from build123d import *

# Parameters (mm, degrees)
SKETCH1_W                         = 120
SKETCH1_H                         = 12
SKETCH2_R                         = 85
BOSS_EXTRUDE1_DEPTH               = 2.5
SKETCH3_R                         = 80
BOSS_EXTRUDE2_DEPTH               = 3
F_12_5_12_5_DIAMETER_HOLE1_D      = 12.5
F_12_5_12_5_DIAMETER_HOLE1_DEPTH  = 14.5
M90_COUNTERBORE_HOLE1_D           = 100
M90_COUNTERBORE_HOLE1_CBORE_D     = 130
M90_COUNTERBORE_HOLE1_CBORE_DEPTH = 1
SKETCH8_R                         = 50.101943112
BOSS_EXTRUDE3_DEPTH               = 7


with BuildPart() as part:
    # Sketch1 → Revolve1 (revolve)
    with BuildSketch(Plane(origin=(0, 234.743963655, 0), x_dir=(1, 0, 0), z_dir=(0, 1, 0))):
        with Locations((581.230642584, 144.692981355)):
            Rectangle(SKETCH1_W, SKETCH1_H)
    revolve(axis=Axis((521.230642584, 234.743963655, -150.692981355), (0, 0, 1)))

    # Sketch2 → Boss-Extrude1 (add)
    with BuildSketch(Plane(origin=(0, 0, -150.692981355), x_dir=(-1, 0, 0), z_dir=(0, 0, -1))):
        with Locations((-521.230642584, 234.743963655)):
            Circle(SKETCH2_R)
    extrude(amount=BOSS_EXTRUDE1_DEPTH)

    # Sketch3 → Boss-Extrude2 (add)
    with BuildSketch(Plane.XY.offset(-138.692981355)):
        with Locations((521.230642584, 234.743963655)):
            Circle(SKETCH3_R)
    extrude(amount=BOSS_EXTRUDE2_DEPTH)

    # Ø12.5 (12.5) Diameter Hole1
    with Locations(Plane.XY.offset(-138.692981355)):
        with Locations((521.230642584, 337.243963655), (609.998246472, 285.993963655), (432.463038696, 285.993963655), (432.463038696, 183.493963655), (521.230642584, 132.243963655), (609.998246472, 183.493963655)):
            Hole(F_12_5_12_5_DIAMETER_HOLE1_D / 2, depth=F_12_5_12_5_DIAMETER_HOLE1_DEPTH)

    # M90 counterbore hole1 (through all)
    with Locations(Plane(origin=(0, 0, -153.192981355), x_dir=(-1, 0, 0), z_dir=(0, 0, -1))):
        with Locations((-521.230642584, 234.743963655)):
            CounterBoreHole(M90_COUNTERBORE_HOLE1_D / 2, M90_COUNTERBORE_HOLE1_CBORE_D / 2, M90_COUNTERBORE_HOLE1_CBORE_DEPTH)

    # Sketch8 → Boss-Extrude3 (add)
    with BuildSketch(Plane.XY.offset(-135.692981355)):
        with Locations((521.230642584, 234.743963655)):
            Circle(SKETCH8_R)
    extrude(amount=-BOSS_EXTRUDE3_DEPTH)


solid = part.part
Design review of the part built by this model. Coordinates are the model's own, in mm. A direction names the side the tool comes from. Coordinates: 2 decimals unless noted, no trailing zeros. Order: outer loops, then holes, each group sorted by start corner. A loop starts at its lowest first (then second) coordinate and runs counter-clockwise, first axis right, second up.
Item 1: For pin 1 Ø5 at (x, z) = (615.5, -146) entering from +Y; pin 2 Ø20 at (x, y) = (521.23, 337.24) entering from +Z; pin 3 Ø1 at (x, z) = (532.5, -140) entering from +Y, all flat-tipped, find the tip position at first contact; note any pin that passes through.
Item 2: For line 1 (X direction, y = 236.5, z = -152); line 2 (Z direction, x = 508, y = 244); line 3 (Z direction, x = 540, y = 291), list the stretches that pass through material, from the lowest coordinate up.
Item 3: The part is to be moulded in two halves that separate along Y. For faces 4 (the cylindrical face through (491.237, 177.078, -152.7)), 5 (the cylindrical face through (401.347, 240.02, -144.777)), 6 (the flat face through (520, 236, -135.693)), 7 (the cylindrical face through (429.1, 291.26, -144.78)), say which applies: pulls with the +Y half, pulls with the -Y half, needs draft (parallel to the pull), parting line crosses it, or undercut.
Item 4: Take a section at B-B, the plane z = -147.5. Write out the cut boundary in (x, y), then the cut area to 3 significant figures.
Item 5: Take a section at D-D, the plane y = 162. Write out the cut boundary in (x, z), then the cut area to 3 significant figures.
Item 6: For faces 1 (the flat face through (521, 235, -142.693)), 2 (the cylindrical face through (441.308, 238.261, -137.214)), 3 (the cylindrical face through (515.27, 339.12, -144.78)), list the 3-axis set-ups (+Z, -Z, +X, -X, +Y, -Y) from which the entire face can be reached by the end or side of a thin tool; tool diameter is ignored.
Item 7: Take a section at C-C, the plane x = 459. Write out the cut boundary in (y, z), then the cut area to 3 significant figures.
Item 8: Take a section at A-A, the plane x = 522. Write out the cut boundary in (y, z), then the cut area to 3 significant figures.
The answers:
1. pin 1: stops at y = 312.06
1. pin 2: stops at z = -138.69
1. pin 3: stops at y = 354.26
2. line 1: x = 436.25 to 471.26, 571.2 to 606.21
2. line 2: z = -142.69 to -135.69
2. line 3: z = -152.19 to -135.69
3. face 4: undercut
3. face 5: parting line crosses it
3. face 6: needs draft
3. face 7: undercut
4. outline: circle Ø240 at (521.23, 234.74); hole circle Ø12.5 at (432.46, 183.49); hole circle Ø12.5 at (432.46, 285.99); hole circle Ø100 at (521.23, 234.74); hole circle Ø12.5 at (521.23, 132.24); hole circle Ø12.5 at (521.23, 337.24); hole circle Ø12.5 at (610, 183.49); hole circle Ø12.5 at (610, 285.99)
4. area: 36,600 mm2
5. outline: (425.79, -150.69) - (477.26, -150.69) - (477.26, -153.19) - (565.2, -153.19) - (565.2, -150.69) - (616.67, -150.69) - (616.67, -138.69) - (554.52, -138.69) - (554.52, -135.69) - (487.94, -135.69) - (487.94, -138.69) - (425.79, -138.69) - close
5. area: 2,710 mm2
6. face 1: -Z
6. face 2: +Z
6. face 3: +Z, -Z
7. outline: (132.14, -150.69) - (176.84, -150.69) - (176.84, -153.19) - (215.97, -153.19) - (215.97, -152.19) - (253.51, -152.19) - (253.51, -153.19) - (292.64, -153.19) - (292.64, -150.69) - (337.35, -150.69) - (337.35, -138.69) - (285.02, -138.69) - (285.02, -135.69) - (184.47, -135.69) - (184.47, -138.69) - (132.14, -138.69) - close
7. area: 3,020 mm2
8. outline: (114.75, -150.69) - (126.04, -150.69) - (126.04, -138.69) - (114.75, -138.69) - close; (138.45, -150.69) - (149.75, -150.69) - (149.75, -153.19) - (169.75, -153.19) - (169.75, -152.19) - (184.75, -152.19) - (184.75, -142.69) - (284.74, -142.69) - (284.74, -152.19) - (299.74, -152.19) - (299.74, -153.19) - (319.74, -153.19) - (319.74, -150.69) - (331.04, -150.69) - (331.04, -138.69) - (314.74, -138.69) - (314.74, -135.69) - (154.75, -135.69) - (154.75, -138.69) - (138.45, -138.69) - close; (343.45, -150.69) - (354.74, -150.69) - (354.74, -138.69) - (343.45, -138.69) - close
8. area: 2,410 mm2
